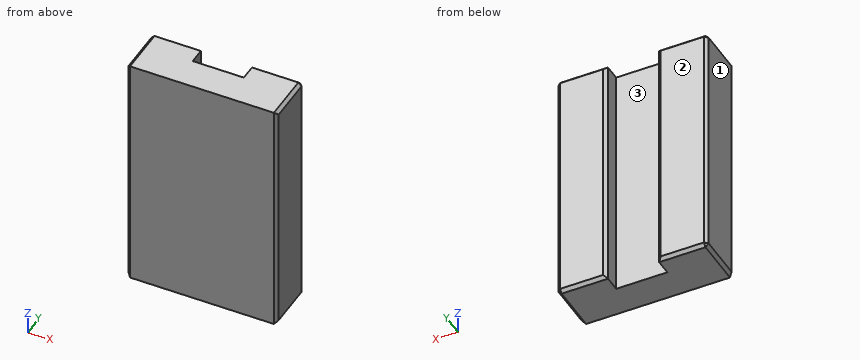
```python
from build123d import *

# Parameters (mm, degrees)
BOSS_EXTRUDE1_DEPTH = 38
CHAMFER1_SIZE       = 0.5


with BuildPart() as part:
    # Sketch1 → Boss-Extrude1 (new body)
    with BuildSketch(Plane.XY):
        Polygon((-11.75, 4), (-4, 4), (-4, 1), (4, 1), (4, 4), (11.75, 4), (11.75, -4), (-11.75, -4), align=None)
    extrude(amount=BOSS_EXTRUDE1_DEPTH)

    # Chamfer1
    chamfer1_edges = [part.edges().sort_by_distance(p)[0] for p in [
        (7.875, 4, 0),
        (11.75, 0, 0),
        (11.75, -4, 19),
        (-11.75, -4, 19),
        (-11.75, 4, 19),
        (-4, 4, 19),
        (4, 4, 19),
        (11.75, 4, 19),
        (-7.875, 4, 38),
        (-11.75, 0, 38),
        (11.75, 0, 38),
        (7.875, 4, 38),
        (-11.75, 0, 0),
        (-7.875, 4, 0),
    ]]
    chamfer(chamfer1_edges, length=CHAMFER1_SIZE)


solid = part.part
```
Read the model definition and answer for the solid it produces. Units are mm, in the model's axes. Face numbers are marked on the shaded views. Coordinates: 2 decimals unless noted, no trailing zeros. Loops run counter-clockwise (first coordinate to the right, second up) from the corner with the lowest first, then second, coordinate; pieces in that order, holes last.
(1) The part is cut by section B-B (z = 17.5). Determine the outline of the cut face in (x, y), and give its area (3 significant figures).
Solution:
outline: (-11.75, -3.5) - (-11.25, -4) - (11.25, -4) - (11.75, -3.5) - (11.75, 3.5) - (11.25, 4) - (4.5, 4) - (4, 3.5) - (4, 1) - (-4, 1) - (-4, 3.5) - (-4.5, 4) - (-11.25, 4) - (-11.75, 3.5) - close
area: 163 mm2
(2) A flat-ended cylindrical pin translates along its axis: pin 1 Ø6.5 at (x, z) = (0, 20) entering from +Y. Find the tip coordinate at first contact, or state that the pin passes through.
Solution:
pin 1: stops at y = 1
(3) The part is cut by section C-C (x = -2). Determine the outline of the cut face in (y, z), and give its area (3 significant figures).
Solution:
outline: (-4, 0) - (1, 0) - (1, 38) - (-4, 38) - close
area: 190 mm2
(4) Consider line 1 along X through (y, z) = (2.5, 32); line 2 along Y through (x, z) = (2, 4). Determine where each line is inside the solid, lowest interval first.
Solution:
line 1: x = -11.75 to -4, 4 to 11.75
line 2: y = -4 to 1
(5) The part is cut by section A-A (y = 2.75). Determine the outline of the cut face in (x, z).
Solution:
outline: (-11.75, 0.5) - (-11.25, 0) - (-4, 0) - (-4, 38) - (-11.25, 38) - (-11.75, 37.5) - close; (4, 0) - (11.25, 0) - (11.75, 0.5) - (11.75, 37.5) - (11.25, 38) - (4, 38) - close
(6) The mould has two halves that part along X. Classify the marked faces 1, 2 and 3: released by +X, released by -X, zero draft, split by the parting line, or undercut.
Solution:
face 1: released by -X
face 2: zero draft
face 3: undercut
